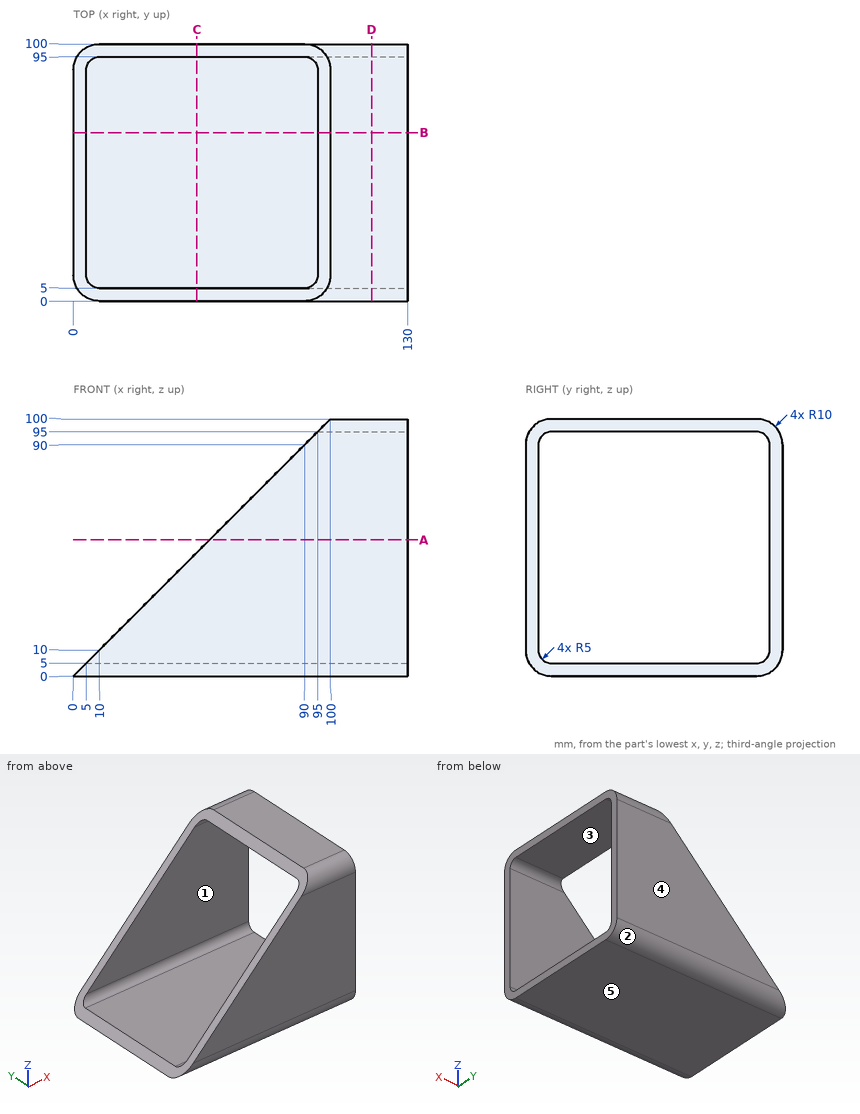
Geometry check sheet. Reference: drawing and pictorial views, mm from the part's lowest x, y, z. A direction names the side the tool comes from. Coordinates: 2 decimals unless noted, no trailing zeros. Order: outer loops, then holes, each group sorted by start corner. A loop starts at its lowest first (then second) coordinate and runs counter-clockwise, first axis right, second up. Notation, with made-up numbers: (22, 73.5) - (62, 73.5) arc R17 cw to (62, 86.5) - close; hole circle Ø2 at (-26.75, 22.25). An arc over 180 degrees is marked (long way). Answer in a Markdown table with one row per item. Add a question column.
1) Cross-section at B-B, the plane y = 65.5. Record the cut outline in (x, z), then the cut area to 3 significant figures.
2) Material ranges on line 1 along Z through (x, y) = (110, 88); line 2 along Z through (x, y) = (30.5, 57), recorded low to high. Write a range as [from, to].
3) Cross-section at C-C, the plane x = 48. Record the cut outline in (y, z), then the cut area to 3 significant figures.
4) Gauge pin test, flat ends, axial feed: P1, Ø6, axis at x = 88, y = 29, coming from the -Z side; P2, Ø1.5, axis at x = 14.5, y = 48, coming from the +Z side. Record the tip position at first contact, or that the pin passes through.
5) Cross-section at D-D, the plane x = 116. Record the cut outline in (y, z).
6) Release check for a two-part mould opening along Z. For the marked faces 3, 4 and 5 record: +Z half, -Z half, draft (parallel to the pull), parting line (faces both ways), or undercut.
7) Set-up check for the marked faces 1 and 2: record each of +Z, -Z, +X, -X, +Y, -Y from which the full face is reachable in a straight line by a thin tool's end or side.
8) Cross-section at A-A, the plane z = 53. Record the cut outline in (x, y).
Check result:
| question | item | result |
|---|---|---|
| 1 | outline | (0, 0) - (130, 0) - (130, 5) - (5, 5) - close; (95, 95) - (130, 95) - (130, 100) - (100, 100) - close |
| 1 | area | 800 mm² |
| 2 | line 1 | z = [0, 5], [95, 100] |
| 2 | line 2 | z = [0, 5] |
| 3 | outline | (0, 10) arc R10 ccw to (10, 0) - (90, 0) arc R10 ccw to (100, 10) - (100, 48) - (95, 48) - (95, 10) arc R5 cw to (90, 5) - (10, 5) arc R5 cw to (5, 10) - (5, 48) - (0, 48) - close |
| 3 | area | 898 mm² |
| 4 | P1 | stops at z = 0 |
| 4 | P2 | stops at z = 5 |
| 5 | outline | (0, 10) arc R10 ccw to (10, 0) - (90, 0) arc R10 ccw to (100, 10) - (100, 90) arc R10 ccw to (90, 100) - (10, 100) arc R10 ccw to (0, 90) - close; hole (5, 10) arc R5 ccw to (10, 5) - (90, 5) arc R5 ccw to (95, 10) - (95, 90) arc R5 ccw to (90, 95) - (10, 95) arc R5 ccw to (5, 90) - close |
| 6 | face 3 | undercut |
| 6 | face 4 | draft |
| 6 | face 5 | -Z half |
| 7 | face 1 | +X, -X |
| 7 | face 2 | -Z, +X, -X, +Y |
| 8 | outline | (53, 0) - (130, 0) - (130, 5) - (53, 5) - close; (53, 95) - (130, 95) - (130, 100) - (53, 100) - close |
